Geometry check sheet. Reference: the model listing, model coordinates, mm. Round coordinates to 2 decimals unless told otherwise and drop trailing zeros. Answer in a Markdown table with one row per item. Add a question column.
```python
from build123d import *

# Parameters (mm, degrees)
SKETCH_1_R      = 2.1
SKETCH_1_R_2    = 3.4
EXTRUDE_1_DEPTH = 630


with BuildPart() as part:
    # 草图1 → 拉伸1 (new body)
    with BuildSketch(Plane(origin=(0, 0, 0), x_dir=(1, 0, 0), z_dir=(0, 1, 0))):
        with BuildLine():
            Line((6.75, -28), (11, -28))
            Line((11, -28), (11, -30))
            Line((11, -30), (2, -30))
            ThreePointArc((2, -30), (0.585786438, -29.414213562), (0, -28))
            Line((0, -28), (0, -19))
            Line((0, -19), (2, -19))
            Line((2, -19), (2, -23.25))
            Line((2, -23.25), (5.335785999, -23.25))
            Line((5.335785999, -23.25), (9, -19.585785999))
            Line((9, -19.585785999), (9, -10.414214001))
            Line((9, -10.414214001), (5.335785999, -6.75))
            Line((5.335785999, -6.75), (2, -6.75))
            Line((2, -6.75), (2, -11))
            Line((2, -11), (0, -11))
            Line((0, -11), (0, -2))
            ThreePointArc((0, -2), (0.585786438, -0.585786438), (2, 0))
            Line((2, 0), (11, 0))
            Line((11, 0), (11, -2))
            Line((11, -2), (6.75, -2))
            Line((6.75, -2), (6.75, -5.335785999))
            Line((6.75, -5.335785999), (10.414214001, -9))
            Line((10.414214001, -9), (19.585785999, -9))
            Line((19.585785999, -9), (23.25, -5.335785999))
            Line((23.25, -5.335785999), (23.25, -2))
            Line((23.25, -2), (19, -2))
            Line((19, -2), (19, 0))
            Line((19, 0), (28, 0))
            ThreePointArc((28, 0), (29.414213562, -0.585786438), (30, -2))
            Line((30, -2), (30, -11))
            Line((30, -11), (28, -11))
            Line((28, -11), (28, -6.75))
            Line((28, -6.75), (24.664214001, -6.75))
            Line((24.664214001, -6.75), (21, -10.414214001))
            Line((21, -10.414214001), (21, -19.585785999))
            Line((21, -19.585785999), (24.664214001, -23.25))
            Line((24.664214001, -23.25), (28, -23.25))
            Line((28, -23.25), (28, -19))
            Line((28, -19), (30, -19))
            Line((30, -19), (30, -28))
            ThreePointArc((30, -28), (29.414213562, -29.414213562), (28, -30))
            Line((28, -30), (19, -30))
            Line((19, -30), (19, -28))
            Line((19, -28), (23.25, -28))
            Line((23.25, -28), (23.25, -24.664214001))
            Line((23.25, -24.664214001), (19.585785999, -21))
            Line((19.585785999, -21), (10.414214001, -21))
            Line((10.414214001, -21), (6.75, -24.664214001))
            Line((6.75, -24.664214001), (6.75, -28))
        make_face()
        with Locations(Location((3.375, -26.625, 0), (0, 0, 270))):
            Circle(SKETCH_1_R, mode=Mode.SUBTRACT)
        with Locations(Location((26.625, -26.625, 0), (0, 0, 270))):
            Circle(SKETCH_1_R, mode=Mode.SUBTRACT)
        with Locations(Location((15, -15, 0), (0, 0, 270))):
            Circle(SKETCH_1_R_2, mode=Mode.SUBTRACT)
        with Locations(Location((3.375, -3.375, 0), (0, 0, 270))):
            Circle(SKETCH_1_R, mode=Mode.SUBTRACT)
        with Locations(Location((26.625, -3.375, 0), (0, 0, 270))):
            Circle(SKETCH_1_R, mode=Mode.SUBTRACT)
    extrude(amount=EXTRUDE_1_DEPTH)


solid = part.part
```
1) Thickness scan on L1, parallel to Z at x = 10.75, y = 392; L2, parallel to Z at x = 27, y = 170; L3, parallel to X at y = 231, z = 15. Record the ranges inside material, lowest first. Write a range as [from, to].
2) Go/stop test with flat-tipped pins: pin 1 (1 mm diameter, centred on y = 202, z = 29, fed in from +X); pin 2 (1 mm diameter, centred on x = 14.5, y = 201.5, fed in from +Z); pin 3 (1 mm diameter, centred on x = 0.5, y = 290.5, fed in from +Z). Record where each tip stops, or that it passes through.
3) Cross-section at A-A, the plane y = 332. Count the separate pieces of the cut face and the enclosed holes in it, plus the area to 3 significant figures.
Worked answers:
| question | item | result |
|---|---|---|
| 1 | L1 | z = [0, 2], [9, 21], [28, 30] |
| 1 | L2 | z = [0, 1.31], [5.44, 6.75], [23.25, 24.56], [28.69, 30] |
| 1 | L3 | x = [9, 11.6], [18.4, 21] |
| 2 | pin 1 | stops at x = 29.94 |
| 2 | pin 2 | stops at z = 21 |
| 2 | pin 3 | stops at z = 29.73 |
| 3 | separate pieces | 1 |
| 3 | enclosed holes | 5 |
| 3 | area | 333 mm2 |
